Could you check a few things on this drawing? It's one solid part, dimensions in mm from its lowest x, y, z. A direction names the side the tool comes from. Give positions to 0.01 mm unless a question says otherwise; leave off trailing zeros. Loops run counter-clockwise (first coordinate to the right, second up) from the corner with the lowest first, then second, coordinate; pieces in that order, holes last. Notation, with made-up numbers: (-8, 35) -> (-2, 35) arc R32 cw to (-2, 64) -> close; hole circle Ø2 at (38.5, 71). An arc over 180 degrees is marked (long way). Use CSV: the item, a comma, the result in double quotes.
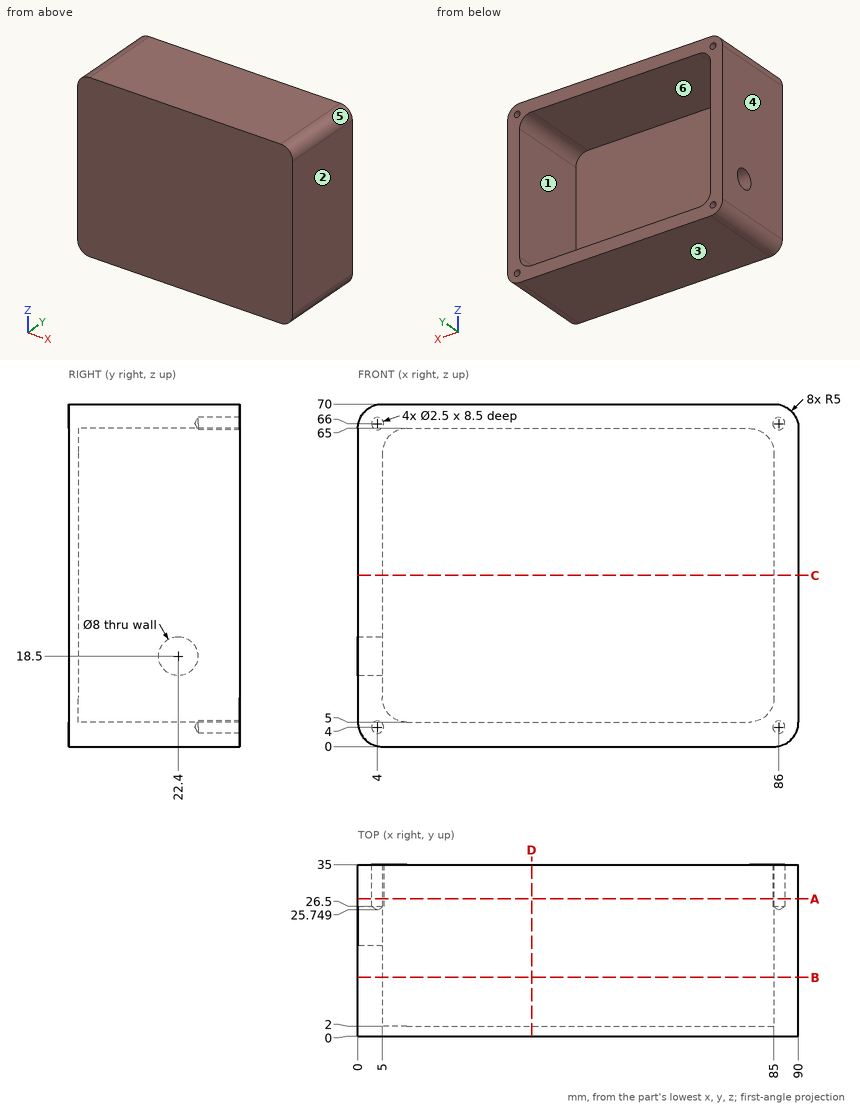
(1) If we section it at D-D, the plane x = 35.5: Write out the boundary of the cut face in (y, z), then the cut area to 3 significant figures.
Answer sheet:
outline,"(0, 0) -> (35, 0) -> (35, 5) -> (2, 5) -> (2, 65) -> (35, 65) -> (35, 70) -> (0, 70) -> close"
area,"470 mm2"
(2) Will these pins go through, and if not, where does the flat tip stop? pin 1 Ø5 at (y, z) = (22.4, 18.5) entering from -X; pin 2 Ø1.5 at (x, z) = (31.5, 28.5) entering from +Y.
Answer sheet:
pin 1,"stops at x = 85"
pin 2,"stops at y = 2"
(3) If we section it at C-C, the plane z = 35: Write out the boundary of the cut face in (x, y), then the cut area to 3 significant figures.
Answer sheet:
outline,"(0, 0) -> (90, 0) -> (90, 35) -> (85, 35) -> (85, 2) -> (5, 2) -> (5, 35) -> (0, 35) -> close"
area,"510 mm2"
(4) We'd pull the mould along X, two halves only. Please class the marked faces 3, 4, 5 and 6: released by +X, released by -X, zero draft, split by the parting line, or undercut.
Answer sheet:
face 3,"zero draft"
face 4,"released by -X"
face 5,"released by +X"
face 6,"undercut"
(5) If we section it at A-A, the plane y = 28: Write out the boundary of the cut face in (x, z).
Answer sheet:
outline,"(0, 5) arc R5 ccw to (5, 0) -> (85, 0) arc R5 ccw to (90, 5) -> (90, 65) arc R5 ccw to (85, 70) -> (5, 70) arc R5 ccw to (0, 65) -> close; hole circle Ø2.5 at (4, 4); hole circle Ø2.5 at (4, 66); hole (5, 10) arc R5 ccw to (10, 5) -> (80, 5) arc R5 ccw to (85, 10) -> (85, 60) arc R5 ccw to (80, 65) -> (10, 65) arc R5 ccw to (5, 60) -> close; hole circle Ø2.5 at (86, 4); hole circle Ø2.5 at (86, 66)"
(6) Which directions (+Z, -Z, +X, -X, +Y, -Y) give clear straight access to the entire face, cutting with the end or side of a thin tool? Please do the marked faces 1 and 2.
Answer sheet:
face 1,"+Y"
face 2,"+Z, -Z, +X, +Y, -Y"
(7) If we section it at B-B, the plane y = 12: Write out the boundary of the cut face in (x, z).
Answer sheet:
outline,"(0, 5) arc R5 ccw to (5, 0) -> (85, 0) arc R5 ccw to (90, 5) -> (90, 65) arc R5 ccw to (85, 70) -> (5, 70) arc R5 ccw to (0, 65) -> close; hole (5, 10) arc R5 ccw to (10, 5) -> (80, 5) arc R5 ccw to (85, 10) -> (85, 60) arc R5 ccw to (80, 65) -> (10, 65) arc R5 ccw to (5, 60) -> close"
(8) If I drill on L1, parallel to Z at x = 53, y = 23; L2, parallel to X at y = 9, z = 29; L3, parallel to Z at x = 86, y = 32.5, over which ranges is the centre line in solid material (lowest first)? Write a range as from..to.
Answer sheet:
L1,"z = 0..5, 65..70"
L2,"x = 0..5, 85..90"
L3,"z = 0.1..2.75, 5.25..64.75, 67.25..69.9"
